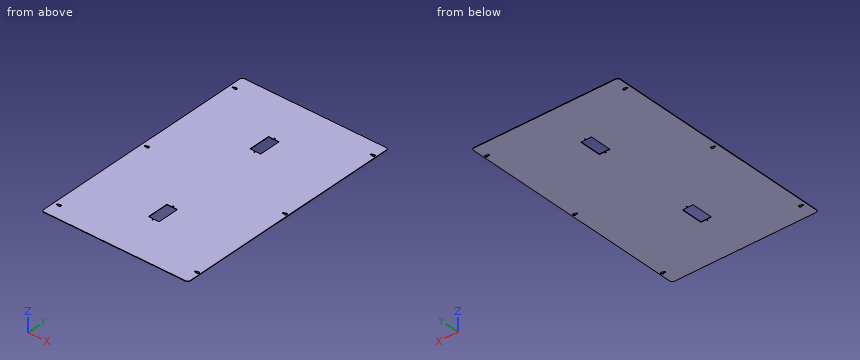
```python
from build123d import *

# Parameters (mm, degrees)
SKETCH1_W            = 615
SKETCH1_H            = 985
BOSS_EXTRUDE1_DEPTH  = 2
SKETCH7_W            = 45
SKETCH7_H            = 91
CUT_EXTRUDE4_DEPTH   = 581.617343868
SKETCH8_R            = 2.25
CUT_EXTRUDE5_DEPTH   = 581.617343868
FILLET3_R            = 10
CUT_EXTRUDE6_DEPTH   = 10
LPATTERN1_COUNT      = 3
LPATTERN1_PITCH      = 432.5
LPATTERN1_COUNT_DIR2 = 2
LPATTERN1_PITCH_DIR2 = 580


with BuildPart() as part:
    # Sketch1 → Boss-Extrude1 (new body)
    with BuildSketch(Plane.XY):
        Rectangle(SKETCH1_W, SKETCH1_H)
    extrude(amount=BOSS_EXTRUDE1_DEPTH)

    # Sketch7 → Cut-Extrude4 (cut, through all)
    with BuildSketch(Plane(origin=(0, 0, 0), x_dir=(-1, 0, 0), z_dir=(0, 0, -1))):
        with Locations((5, 250)):
            Rectangle(SKETCH7_W, SKETCH7_H)
        with Locations((5, -250)):
            Rectangle(SKETCH7_W, SKETCH7_H)
    extrude(amount=-CUT_EXTRUDE4_DEPTH, mode=Mode.SUBTRACT)

    # Sketch8 → Cut-Extrude5 (cut, through all)
    with BuildSketch(Plane(origin=(0, 0, 0), x_dir=(-1, 0, 0), z_dir=(0, 0, -1))):
        with Locations((5, 300)):
            Circle(SKETCH8_R)
        with Locations((5, 200)):
            Circle(SKETCH8_R)
        with Locations((5, -200)):
            Circle(SKETCH8_R)
        with Locations((5, -300)):
            Circle(SKETCH8_R)
    extrude(amount=-CUT_EXTRUDE5_DEPTH, mode=Mode.SUBTRACT)

    # Fillet3
    fillet3_edges = [part.edges().sort_by_distance(p)[0] for p in [
        (307.5, -492.5, 1),
        (-307.5, -492.5, 1),
        (-307.5, 492.5, 1),
        (307.5, 492.5, 1),
    ]]
    fillet(fillet3_edges, radius=FILLET3_R)

    # Sketch10 → Cut-Extrude6 (cut)
    with BuildSketch(Plane(origin=(0, 0, 0), x_dir=(-1, 0, 0), z_dir=(0, 0, -1))):
        with BuildLine():
            Line((292.5, 435.8), (286.9, 435.8))
            ThreePointArc((286.9, 435.8), (277, 432.5), (286.9, 429.2))
            Line((286.9, 429.2), (292.5, 429.2))
            ThreePointArc((292.5, 429.2), (295.8, 432.5), (292.5, 435.8))
        make_face()
    cut_extrude6 = extrude(amount=-CUT_EXTRUDE6_DEPTH, mode=Mode.SUBTRACT)

    # LPattern1: Cut-Extrude6 3 × 2
    with Locations(*[(j * LPATTERN1_PITCH_DIR2, -i * LPATTERN1_PITCH, 0) for i in range(LPATTERN1_COUNT) for j in range(LPATTERN1_COUNT_DIR2) if (i, j) != (0, 0)]):
        add(cut_extrude6, mode=Mode.SUBTRACT)


solid = part.part
```
For this review, take the finished solid that the model builds, in its own axes (mm). Give positions to 0.01 mm unless a question says otherwise; leave off trailing zeros. Write each loop counter-clockwise with the first axis right and the second up, starting at its lowest first coordinate (ties: lowest second). Pieces come first, ordered by that corner, then holes.
Item 1: Take a section at B-B (z = 0.8). Give the number of separate pieces and of enclosed holes in the cut face, and give its area (3 significant figures).
Item 2: Take a section at A-A (y = 270). Give the boundary of the cut face in (x, z), and give its area (3 significant figures).
Item 3: Wall thickness on probe 1 along Y at (x, z) = (297.5, 1.6); probe 2 along X at (y, z) = (0, 1.45); probe 3 along Y at (x, z) = (7, 0.65): over which ranges is each line inside the solid? List them lowest first.
Established:
1. separate pieces: 1
1. enclosed holes: 12
1. area: 597,000 mm2
2. outline: (-307.5, 0) - (-27.5, 0) - (-27.5, 2) - (-307.5, 2) - close; (17.5, 0) - (307.5, 0) - (307.5, 2) - (17.5, 2) - close
2. area: 1,140 mm2
3. probe 1: y = -492.5 to -438, -427 to -5.5, 5.5 to 427, 438 to 492.5
3. probe 2: x = -307.5 to -295.8, -277 to 284.2, 303 to 307.5
3. probe 3: y = -492.5 to -295.5, -204.5 to 204.5, 295.5 to 492.5
